Can you work these out from the model? Positions are in its coordinate system, mm. Give positions to 0.01 mm unless a question says otherwise; leave off trailing zeros. Loops run counter-clockwise (first coordinate to the right, second up) from the corner with the lowest first, then second, coordinate; pieces in that order, holes last. Notation, with made-up numbers: (33.5, 4.25) -> (74.5, 4.25) arc R22 cw to (74.5, 18.25) -> close; hole circle Ø1 at (-29, 36). An arc over 180 degrees is marked (long way). Return JSON: item names as keys, results as strings. Group by question number.
Q1. I need wall thicknesses on line 1 along Y through (x, z) = (0, 4.75); line 2 along Y through (x, z) = (-51.5, 13.25); line 3 along X through (y, z) = (-41, 6.75). Which ranges of each line are inside material? Lowest first, please. Write a range as [from, to].
Q2. Suppose I cut it at C-C, the plane z = 7.5. Please give me the cut outline in (x, y).
Q3. Suppose I cut it at A-A, the plane x = 0. Please give me the cut outline in (y, z).
Q4. Suppose I cut it at B-B, the plane y = 0. Please give me the cut outline in (x, z).
```python
from build123d import *

# Parameters (mm, degrees)
SKETCH_1_W      = 250
SKETCH_1_H      = 350
SKETCH_1_R      = 90
EXTRUDE_1_DEPTH = 16


with BuildPart() as part:
    # 草图1 → 凸台-拉伸1 (new body)
    with BuildSketch(Plane.XY):
        Rectangle(SKETCH_1_W, SKETCH_1_H)
        Circle(SKETCH_1_R, mode=Mode.SUBTRACT)
    extrude(amount=EXTRUDE_1_DEPTH)


solid = part.part
```
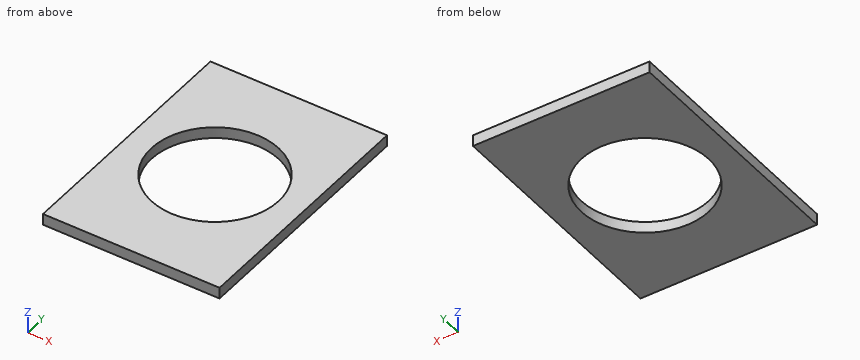
Ans:
{
 "1": {"line 1": "y = [-175, -90], [90, 175]", "line 2": "y = [-175, -73.81], [73.81, 175]", "line 3": "x = [-125, -80.12], [80.12, 125]"},
 "2": {"outline": "(-125, -175) -> (125, -175) -> (125, 175) -> (-125, 175) -> close; hole circle Ø180 at (0, 0)"},
 "3": {"outline": "(-175, 0) -> (-90, 0) -> (-90, 16) -> (-175, 16) -> close; (90, 0) -> (175, 0) -> (175, 16) -> (90, 16) -> close"},
 "4": {"outline": "(-125, 0) -> (-90, 0) -> (-90, 16) -> (-125, 16) -> close; (90, 0) -> (125, 0) -> (125, 16) -> (90, 16) -> close"}
}
